from build123d import *

# Parameters (mm, degrees)
CUT_EXTRUDE1_DEPTH      = 1
CUT_EXTRUDE1_DEPTH_BACK = 35
CUT_EXTRUDE1_START      = 65


with BuildPart() as part:
    # Sketch1 → Revolve1 (revolve)
    with BuildSketch(Plane.XY, mode=Mode.PRIVATE) as revolve1_sk:
        Polygon((0, 0), (0, 25), (60, 25), (60, 35), (157.35, 35), (157.35, 32.35), (160, 32.35), (160, 35), (610, 35), (610, 20), (635.67, 20), (635.67, 17.35), (638.32, 17.35), (638.32, 20), (661.99, 20), (661.99, 15), (691.99, 15), (691.99, 0), align=None)
    revolve(revolve1_sk.sketch.rotate(Axis((0, 0, 0), (1, 0, 0)), 180), axis=Axis((0, 0, 0), (1, 0, 0)))

    # Sketch2 → Cut-Extrude1 (cut, two sides: drawn at the far end of the back side and taken through both)
    with BuildSketch(Plane(origin=(0, 0, 0), x_dir=(1, 0, 0), z_dir=(0, 1, 0)).offset(CUT_EXTRUDE1_START - CUT_EXTRUDE1_DEPTH_BACK)):
        with BuildLine():
            Line((81, 6), (124, 6))
            ThreePointArc((124, 6), (130, 0), (124, -6))
            Line((124, -6), (81, -6))
            ThreePointArc((81, -6), (75, 0), (81, 6))
        make_face()
    extrude(amount=CUT_EXTRUDE1_DEPTH + CUT_EXTRUDE1_DEPTH_BACK, mode=Mode.SUBTRACT)


solid = part.part
Can you work these out from the model? Positions are in its coordinate system, mm. A direction names the side the tool comes from. Give positions to 0.01 mm unless a question says otherwise; leave off trailing zeros. Write each loop counter-clockwise with the first axis right and the second up, starting at its lowest first coordinate (ties: lowest second). Pieces come first, ordered by that corner, then holes. Notation, with made-up numbers: (83.25, 88.25) -> (120.25, 88.25) arc R11 ccw to (120.25, 98.25) -> close; hole circle Ø2 at (-10, -15.5). An arc over 180 degrees is marked (long way). Answer as a JSON object with one key per item and string values. Group by question number.
Item 1: Suppose I cut it at B-B (x = 383.5). Please give me the cut outline in (y, z), plus the area to 3 significant figures.
Item 2: Please list where these lines run through material, in increasing order: line 1 (X direction, y = 22.5, z = 26.5); line 2 (X direction, y = 7, z = -17); line 3 (Y direction, x = 581.5, z = 2.5). Write a range as [from, to].
Item 3: We'd pull the mould along Z, two halves only. Please class faces 4 (the face through (103, 30, 0)), 5 (the face through (610, -15, 15)), 6 (the face through (677.2, -8.06, -12.65)): +Z half, -Z half, draft (parallel to the pull), parting line (faces both ways), or undercut.
Item 4: I'm going to push flat-ended pins straight in: P1, Ø12, axis at x = 603, y = -15.5, coming from the +Z side; P2, Ø2, axis at x = 97.5, z = 24, coming from the -Y side; P3, Ø5, axis at x = 110.5, y = 32, coming from the +Z side; P4, Ø12, axis at x = 508.5, z = 1, coming from the +Y side. Where does each tip first touch, or does it pass through?
Item 5: For faces 1 (the face through (60, -24, -8)), 2 (the face through (650.32, 19.98, -0.88)), 3 (the face through (637.014, 2.259, -17.202)), which set-ups out of +Z, -Z, +X, -X, +Y, -Y let a thin tool reach every point of the face, with its end or its side?
Findings:
{
 "1": {"outline": "circle Ø70 at (0, 0)", "area": "3,850 mm²"},
 "2": {"line 1": "x = [60, 157.35], [160, 610]", "line 2": "x = [0, 635.67], [638.32, 661.99]", "line 3": "y = [-34.91, 34.91]"},
 "3": {"face 4": "undercut", "face 5": "draft", "face 6": "parting line"},
 "4": {"P1": "stops at z = 33.69", "P2": "stops at y = -26.38", "P3": "stops at z = 18.83", "P4": "stops at y = 35"},
 "5": {"face 1": "-X", "face 2": "+X", "face 3": "none"}
}
